CAD build for the part. Positions are in the model's coordinates, mm. Face numbers are marked on the shaded views. A direction names the side the tool comes from. Give positions to 0.01 mm unless a question says otherwise; leave off trailing zeros. Write each loop counter-clockwise with the first axis right and the second up, starting at its lowest first coordinate (ties: lowest second). Pieces come first, ordered by that corner, then holes. Notation, with made-up numbers: (-37, 24.5) - (-3, 24.5) arc R21 cw to (-3, 30.5) - close; hole circle Ø11 at (30.5, 12). An arc over 180 degrees is marked (long way). Answer as a JSON object with one key per item and string values.
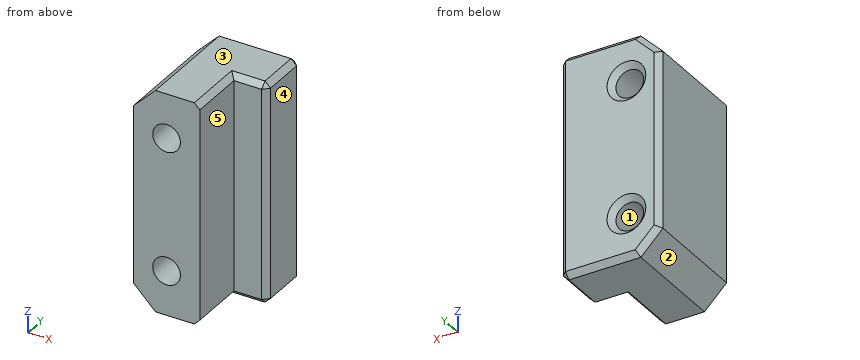
from build123d import *

# Parameters (mm, degrees)
EXTRUDE_1_DEPTH    = 20
HOLE_WIZARD_M3_1_D = 2.5
CHAMFER_1_SIZE     = 2
CHAMFER_2_SIZE     = 0.5


with BuildPart() as part:
    # 草图1 → 凸台-拉伸1 (new body)
    with BuildSketch(Plane.XY):
        Polygon((0, 0), (6, 0), (6, 5.1), (9, 5.1), (9, 10), (0, 10), align=None)
    extrude(amount=EXTRUDE_1_DEPTH)

    # M3 螺纹孔1 (through all)
    with Locations(Plane(origin=(0, 10, 0), x_dir=(1, 0, 0), z_dir=(0, 1, 0))):
        with Locations((3, -16), (3, -4)):
            Hole(HOLE_WIZARD_M3_1_D / 2)

    # 倒角1
    chamfer_1_edges = [part.edges().sort_by_distance(p)[0] for p in [
        (0, 5, 20),
        (0, 5, 0),
    ]]
    chamfer(chamfer_1_edges, length=CHAMFER_1_SIZE)

    # 倒角2
    chamfer_2_edges = [part.edges().sort_by_distance(p)[0] for p in [
        (6, 2.55, 20),
        (9, 10, 10),
        (9, 5.1, 10),
        (7.5, 5.1, 20),
        (0, 10, 10),
        (1, 10, 19),
        (1, 10, 1),
        (9, 7.55, 20),
        (5.5, 10, 20),
        (4.25, 10, 4),
        (4.25, 10, 16),
        (5.5, 10, 0),
        (9, 7.55, 0),
        (7.5, 5.1, 0),
        (6, 2.55, 0),
    ]]
    chamfer(chamfer_2_edges, length=CHAMFER_2_SIZE)


solid = part.part
(1) Saw through at B-B, the plane z = 4. Give the cut face in (x, y).
Answer key:
{"outline": "(0, 0) - (1.75, 0) - (1.75, 9.5) - (1.25, 10) - (0.5, 10) - (0, 9.5) - close; (4.25, 0) - (6, 0) - (6, 5.1) - (8.5, 5.1) - (9, 5.6) - (9, 9.5) - (8.5, 10) - (4.75, 10) - (4.25, 9.5) - close"}
(2) Saw through at A-A, the plane x = 3. Give the cut face in (y, z), and give its area (3 significant figures).
Answer key:
{"outline": "(0, 0) - (9.5, 0) - (10, 0.5) - (10, 2.25) - (9.5, 2.75) - (0, 2.75) - close; (0, 5.25) - (9.5, 5.25) - (10, 5.75) - (10, 14.25) - (9.5, 14.75) - (0, 14.75) - close; (0, 17.25) - (9.5, 17.25) - (10, 17.75) - (10, 19.5) - (9.5, 20) - (0, 20) - close", "area": "149 mm²"}
(3) Flat gauge pins, fed straight in: P1, Ø2.5, axis at y = 2.5, z = 8.5, coming from the +X side; P2, Ø3, axis at x = 3, z = 16, coming from the +Y side. Where does each tip first touch, or does it go through?
Answer key:
{"P1": "stops at x = 6", "P2": "stops at y = 9.75"}
(4) Saw through at C-C, the plane y = 1.75. Give the cut face in (x, z), and give its area (3 significant figures).
Answer key:
{"outline": "(0, 2) - (2, 0) - (5.5, 0) - (6, 0.5) - (6, 19.5) - (5.5, 20) - (2, 20) - (0, 18) - close; hole circle Ø2.5 at (3, 4); hole circle Ø2.5 at (3, 16)", "area": "106 mm²"}
(5) 3-axis set-ups, long thin cutter, end or side, ignore diameter. For the marked faces 4 and 5: which of +Z, -Z, +X, -X, +Y, -Y reach the whole face in a straight line?
Answer key:
{"face 4": "+Z, -Z, +X, +Y, -Y", "face 5": "+Z, -Z, +X, -Y"}
(6) Pull direction X, two halves, no side cores. Call the marked faces 1, 2 and 3: pulls with the +X half, pulls with the -X half, needs draft (parallel to the pull), parting line crosses it, or undercut.
Answer key:
{"face 1": "undercut", "face 2": "pulls with the -X half", "face 3": "needs draft"}
(7) Probe L1, parallel to Z at x = 3, y = 7.25; L2, parallel to X at y = 6.75, z = 16; L3, parallel to X at y = 3.75, z = 16. List the from-to ranges inside material, lowest first. Write a range as [from, to].
Answer key:
{"L1": "z = [0, 2.75], [5.25, 14.75], [17.25, 20]", "L2": "x = [0, 1.75], [4.25, 9]", "L3": "x = [0, 1.75], [4.25, 6]"}
(8) Saw through at D-D, the plane z = 6. Give the cut face in (x, y).
Answer key:
{"outline": "(0, 0) - (6, 0) - (6, 5.1) - (8.5, 5.1) - (9, 5.6) - (9, 9.5) - (8.5, 10) - (0.5, 10) - (0, 9.5) - close"}
